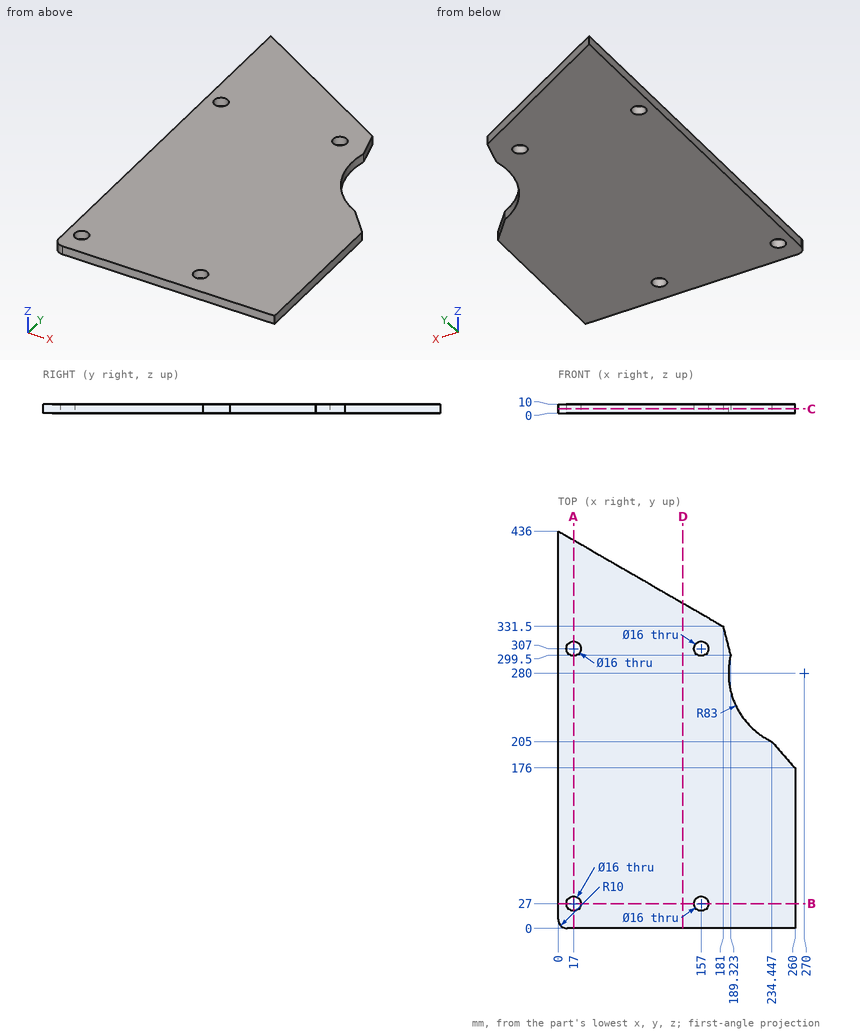
Can you work these out from the drawing? Everything is in mm from the part's minimum corner. Coordinates: 2 decimals unless noted, no trailing zeros. Write each loop counter-clockwise with the first axis right and the second up, starting at its lowest first coordinate (ties: lowest second). Pieces come first, ordered by that corner, then holes. Notation, with made-up numbers: (43.25, 70) -> (47.25, 70) arc R22 ccw to (47.25, 81) -> close; hole circle Ø10 at (-15, 46.5). An arc over 180 degrees is marked (long way). Write each question's results on one line, items separated by ' | '. Start each with the question number.
Item 1: Please list where these lines run through material, in increasing order: probe 1 along X at (y, z) = (30, 6.25) (1 decimal); probe 2 along Y at (x, z) = (157, 5.25) (1 decimal); probe 3 along Y at (x, z) = (17, 7.5) (1 decimal).
Item 2: If we section it at D-D, the plane x = 137: Write out the boundary of the cut face in (y, z).
Item 3: If we section it at B-B, the plane y = 27: Write out the boundary of the cut face in (x, z).
Item 4: If we section it at A-A, the plane x = 17: Write out the boundary of the cut face in (y, z) (1 decimal), and give its area (3 significant figures).
Item 5: I'm going to push flat-ended pins straight in: P1, Ø3, axis at x = 89, y = 205.5, coming from the -Z side; P2, Ø14.5, axis at x = 17, y = 307, coming from the +Z side. Where does each tip first touch, or does it pass through?
Item 6: If we section it at C-C, the plane z = 4.75: Write out the boundary of the cut face in (x, y).
Answer block:
1) probe 1: 0 to 9.6, 24.4 to 149.6, 164.4 to 260 | probe 2: 0 to 19, 35 to 299, 315 to 345.4 | probe 3: 0 to 19, 35 to 299, 315 to 426.2
2) outline: (0, 0) -> (356.9, 0) -> (356.9, 10) -> (0, 10) -> close
3) outline: (0, 0) -> (9, 0) -> (9, 10) -> (0, 10) -> close; (25, 0) -> (149, 0) -> (149, 10) -> (25, 10) -> close; (165, 0) -> (260, 0) -> (260, 10) -> (165, 10) -> close
4) outline: (0, 0) -> (19, 0) -> (19, 10) -> (0, 10) -> close; (35, 0) -> (299, 0) -> (299, 10) -> (35, 10) -> close; (315, 0) -> (426.2, 0) -> (426.2, 10) -> (315, 10) -> close | area: 3,940 mm²
5) P1: z = 0 | P2: through
6) outline: (0, 10) arc R10 ccw to (10, 0) -> (260, 0) -> (260, 176) -> (234.45, 205) arc R83 cw to (189.32, 299.5) -> (181, 331.5) -> (0, 436) -> close; hole circle Ø16 at (17, 27); hole circle Ø16 at (17, 307); hole circle Ø16 at (157, 27); hole circle Ø16 at (157, 307)
